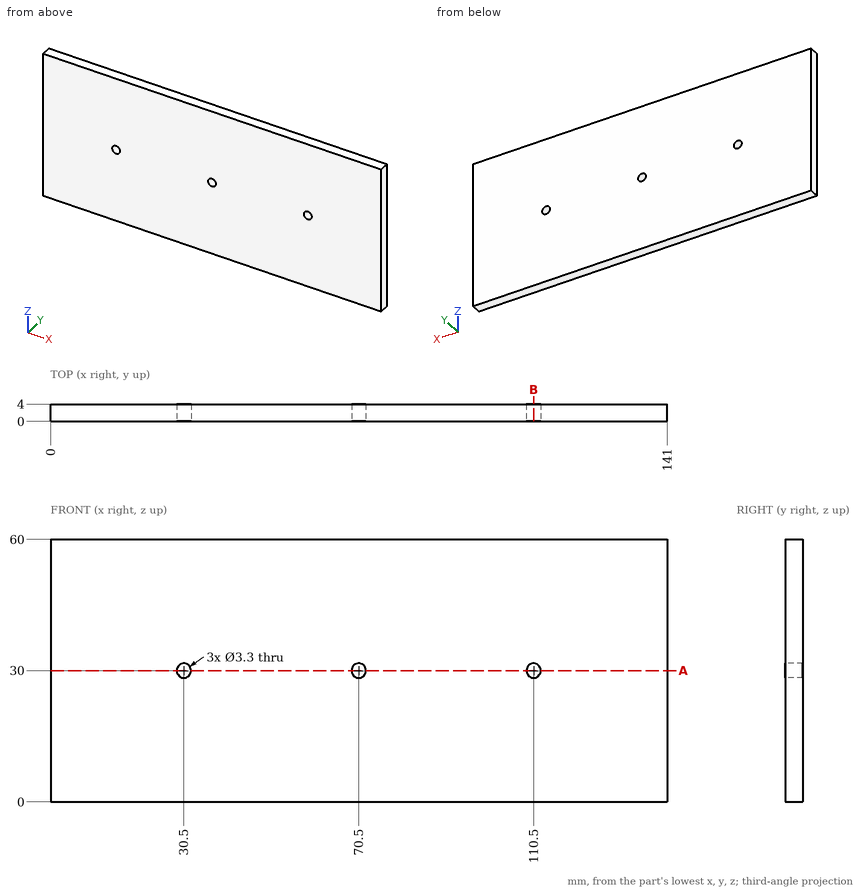
Here's the drawing with two shaded views (mm, measured from the low corner). I have some questions. Round coordinates to 2 decimals unless told otherwise and drop trailing zeros. Loops run counter-clockwise (first coordinate to the right, second up) from the corner with the lowest first, then second, coordinate; pieces in that order, holes last. Notation, with made-up numbers: (-4.75, 73) - (20.25, 73) arc R24 ccw to (20.25, 93) - close; hole circle Ø10 at (80, 4). An arc over 180 degrees is marked (long way). Write item = value, one per line.
1) Imagine slicing it at A-A (z = 30). Please give me the cut outline in (x, y), and give its area (3 significant figures).
Computed:
outline = (0, 0) - (28.85, 0) - (28.85, 4) - (0, 4) - close; (32.15, 0) - (68.85, 0) - (68.85, 4) - (32.15, 4) - close; (72.15, 0) - (108.85, 0) - (108.85, 4) - (72.15, 4) - close; (112.15, 0) - (141, 0) - (141, 4) - (112.15, 4) - close
area = 524 mm2
2) Imagine slicing it at B-B (x = 110.5). Please give me the cut outline in (y, z).
Computed:
outline = (0, 0) - (4, 0) - (4, 28.35) - (0, 28.35) - close; (0, 31.65) - (4, 31.65) - (4, 60) - (0, 60) - close
3) I need wall thicknesses on line 1 along X through (y, z) = (3.2, 30); line 2 along Z through (x, y) = (30.5, 2.55); line 3 along X through (y, z) = (0.5, 29). Which ranges of each line are inside material? Lowest first, please. Write a range as from..to.
Computed:
line_1 = 0..28.85, 32.15..68.85, 72.15..108.85, 112.15..141
line_2 = 0..28.35, 31.65..60
line_3 = 0..29.19, 31.81..69.19, 71.81..109.19, 111.81..141
